Input: part model. Units: mm. Frame: model coordinates. Face numbers are marked on the shaded views. A direction names the side the tool comes from. Give positions to 0.01 mm unless a question says otherwise; leave off trailing zeros. Loops run counter-clockwise (first coordinate to the right, second up) from the corner with the lowest first, then second, coordinate; pieces in that order, holes last. Notation, with made-up numbers: (67, -27.75) - (107, -27.75) arc R8 cw to (107, -20.75) - close; hole circle Ø4 at (33.5, 45). An arc over 180 degrees is marked (long way). One line per question, with ' | ' between items. Start each with the question number.
from build123d import *

# Parameters (mm, degrees)
CUT_EXTRUDE_1_DEPTH = 4
SKETCH_3_R          = 15
SKETCH_3_R_2        = 14.3
CUT_EXTRUDE_2_DEPTH = 1.3


with BuildPart() as part:
    # 草图1 → 旋转1 (revolve)
    with BuildSketch(Plane.XY):
        Polygon((0, 0), (0, 20), (60, 20), (60, 23), (130, 23), (130, 20), (197.7, 20), (197.7, 15), (280.7, 15), (280.7, 0), align=None)
    revolve(axis=Axis((280.7, 0, 0), (-1, 0, 0)))

    # 草图2 → 切除-拉伸1 (cut)
    with BuildSketch(Plane(origin=(0, 15, 0), x_dir=(1, 0, 0), z_dir=(0, 1, 0))):
        with BuildLine():
            Line((207.7, 4), (290.7, 4))
            Line((290.7, 4), (290.7, -4))
            Line((290.7, -4), (207.7, -4))
            ThreePointArc((207.7, -4), (203.7, 0), (207.7, 4))
        make_face()
    extrude(amount=-CUT_EXTRUDE_1_DEPTH, mode=Mode.SUBTRACT)

    # 草图3 → 切除-拉伸2 (cut)
    with BuildSketch(Plane(origin=(270.9, 0, 0), x_dir=(0, 0, -1), z_dir=(1, 0, 0))):
        with Locations(Location((0, 0, 0), (0, 0, 90))):
            Circle(SKETCH_3_R)
        Circle(SKETCH_3_R_2, mode=Mode.SUBTRACT)
    extrude(amount=-CUT_EXTRUDE_2_DEPTH, mode=Mode.SUBTRACT)


solid = part.part
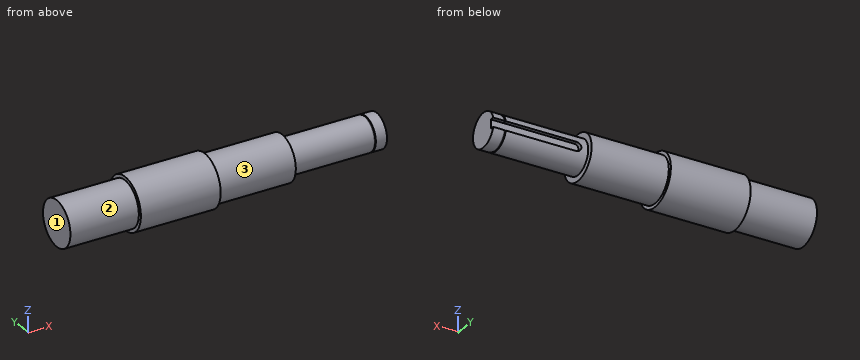
Q1. Section B-B, the plane y = 0. Output: boundary loops of the cut face in (x, z).
Q2. Section D-D, the plane y = -11.5. Output: boundary loops of the cut face in (x, z), plus the area to 3 significant figures.
Q3. Line query: L1, parallel to X at y = -3, z = -14.5; L2, parallel to Y at x = 38, z = -14; L3, parallel to X at y = -9.5, z = -20. Output: solid intervals per line, ascending. Write a range as from..to.
Q4. Access query for the marked faces 1, 2 and 3. Directions: +Z, -Z, +X, -X, +Y, -Y. A direction counts if a zero-diameter tool reaches every point of the face in a straight line with its end or side. Return the directions, or none.
Q5. First-contact query: pin 1 (12 mm diameter, centred on x = 58.5, z = 9.5, fed in from -Y); pin 2 (1.5 mm diameter, centred on x = 149, z = 12.5, fed in from -Y); pin 3 (5 mm diameter, centred on x = 36.5, y = -13, fed in from -Z). Flat tips, straight axial feed; report the tip coordinate or a pass-through.
Q6. Section A-A, the plane z = 0. Output: boundary loops of the cut face in (x, y), plus the area to 3 significant figures.
Q7. Section C-C, the plane x = 57.5. Output: boundary loops of the cut face in (y, z).
Solved:
1) outline: (0, -20) - (60, -20) - (60, -23) - (130, -23) - (130, -20) - (197.7, -20) - (197.7, -15) - (269.6, -15) - (269.6, -14.3) - (270.9, -14.3) - (270.9, -15) - (280.7, -15) - (280.7, 15) - (270.9, 15) - (270.9, 14.3) - (269.6, 14.3) - (269.6, 15) - (197.7, 15) - (197.7, 20) - (130, 20) - (130, 23) - (60, 23) - (60, 20) - (0, 20) - close
2) outline: (0, -16.36) - (60, -16.36) - (60, -19.92) - (130, -19.92) - (130, -16.36) - (197.7, -16.36) - (197.7, -9.63) - (269.6, -9.63) - (269.6, -8.5) - (270.9, -8.5) - (270.9, -9.63) - (280.7, -9.63) - (280.7, 9.63) - (270.9, 9.63) - (270.9, 8.5) - (269.6, 8.5) - (269.6, 9.63) - (197.7, 9.63) - (197.7, 16.36) - (130, 16.36) - (130, 19.92) - (60, 19.92) - (60, 16.36) - (0, 16.36) - close | area: 8,560 mm²
3) L1: x = 0..269.6, 270.9..280.7 | L2: y = -14.28..14.28 | L3: x = 60..130
4) face 1: +Z, -Z, -X, +Y, -Y | face 2: -X | face 3: +X
5) pin 1: stops at y = -22.7 | pin 2: stops at y = -16.18 | pin 3: stops at z = -17.02
6) outline: (0, -20) - (60, -20) - (60, -23) - (130, -23) - (130, -20) - (197.7, -20) - (197.7, -15) - (269.6, -15) - (269.6, -14.3) - (270.9, -14.3) - (270.9, -15) - (280.7, -15) - (280.7, 11) - (203.7, 11) - (203.7, 15) - (197.7, 15) - (197.7, 20) - (130, 20) - (130, 23) - (60, 23) - (60, 20) - (0, 20) - close | area: 10,500 mm²
7) outline: circle Ø40 at (0, 0)
